Can you work these out from the model? Positions are in its coordinate system, mm. Round coordinates to 2 decimals unless told otherwise and drop trailing zeros. Order: outer loops, then holes, each group sorted by start corner. A loop starts at its lowest first (then second) coordinate and runs counter-clockwise, first axis right, second up. Notation, with made-up numbers: M 28,33 L 52,33 A17 cw 52,43 Z; hole C 79.5,-19 d2. An arc over 180 degrees is marked long. Answer as a JSON object with one key per item and string values. Group by question number.
from build123d import *

# Parameters (mm, degrees)
BOSS_EXTRUDE1_DEPTH   = 15
M8_TAPPED_HOLE1_D     = 6.8
M8_TAPPED_HOLE1_DEPTH = 19.75
M8_TAPPED_HOLE1_TIP   = 2.042926105


with BuildPart() as part:
    # Sketch1 → Boss-Extrude1 (new body)
    with BuildSketch(Plane.XY):
        Polygon((-37.5, 32.5), (-32.5, 37.5), (32.5, 37.5), (37.5, 32.5), (37.5, -32.5), (32.5, -37.5), (-32.5, -37.5), (-37.5, -32.5), align=None)
    extrude(amount=BOSS_EXTRUDE1_DEPTH)

    # M8 Tapped Hole1
    with Locations(Plane.XY.offset(15)):
        with Locations((-29, 27.5), (29, 27.5), (29, -27.5), (-29, -27.5)):
            Hole(M8_TAPPED_HOLE1_D / 2, depth=M8_TAPPED_HOLE1_DEPTH)
            with Locations((0, 0, -(M8_TAPPED_HOLE1_DEPTH + M8_TAPPED_HOLE1_TIP / 2))):  # 118° drill point
                Cone(0, M8_TAPPED_HOLE1_D / 2, M8_TAPPED_HOLE1_TIP, mode=Mode.SUBTRACT)


solid = part.part
Item 1: Suppose I cut it at C-C, the plane z = 6.5. Write out the boundary of the cut face in (x, y), and give its area (3 significant figures).
Item 2: Suppose I cut it at B-B, the plane x = -29. Write out the boundary of the cut face in (y, z), and give its area (3 significant figures).
Item 3: Suppose I cut it at A-A, the plane y = -27.5. Write out the boundary of the cut face in (x, z).
Item 4: I need wall thicknesses on line 1 (Y direction, x = 29, z = 5). Which ranges of the line are inside material? Lowest first, please.
Item 5: I'm going to push flat-ended pins straight in: pin 1 Ø8 at (x, y) = (-29, -27.5) entering from -Z; pin 2 Ø6 at (x, y) = (29, -27.5) entering from +Z. Where does each tip first touch, or does it pass through?
Item 6: If we mould it in two halves opening along X, with no side actions, what happens to faces 1 (the face through (0, -37.5, 7)), 2 (the face through (-32.14, -28.8, 7.4)), 3 (the face through (-37.5, 0, 7))? For each: +X half, -X half, draft (parallel to the pull), parting line (faces both ways), or undercut.
Computed:
{
 "1": {"outline": "M -37.5,-32.5 L -32.5,-37.5 L 32.5,-37.5 L 37.5,-32.5 L 37.5,32.5 L 32.5,37.5 L -32.5,37.5 L -37.5,32.5 Z; hole C -29,-27.5 d6.8; hole C -29,27.5 d6.8; hole C 29,-27.5 d6.8; hole C 29,27.5 d6.8", "area": "5,430 mm^2"},
 "2": {"outline": "M -37.5,0 L -30.9,0 L -30.9,15 L -37.5,15 Z; M -24.1,0 L 24.1,0 L 24.1,15 L -24.1,15 Z; M 30.9,0 L 37.5,0 L 37.5,15 L 30.9,15 Z", "area": "921 mm^2"},
 "3": {"outline": "M -37.5,0 L -32.4,0 L -32.4,15 L -37.5,15 Z; M -25.6,0 L 25.6,0 L 25.6,15 L -25.6,15 Z; M 32.4,0 L 37.5,0 L 37.5,15 L 32.4,15 Z"},
 "4": {"line 1": "y = -37.5 to -30.9, -24.1 to 24.1, 30.9 to 37.5"},
 "5": {"pin 1": "stops at z = 0", "pin 2": "passes through"},
 "6": {"face 1": "draft", "face 2": "undercut", "face 3": "-X half"}
}
